from build123d import *

# Parameters (mm, degrees)
BASE_BLOCK_SKETCH_W     = 90
BASE_BLOCK_SKETCH_H     = 33
BASE_BLOCK_DEPTH        = 32
BOTTOM_SLOT_SKETCH_W    = 26
BOTTOM_SLOT_SKETCH_H    = 14
BOTTOM_SLOT_DEPTH       = 102.05938848
SUPPORT_UPRIGHTS_DEPTH  = 90
CENTRE_RECESS_DEPTH     = 128.027556066
CRADLE_ARC_CUT_DEPTH    = 128.027556066
UPRIGHT_U_SLOT_SKETCH_W = 28
UPRIGHT_U_SLOT_SKETCH_H = 16
UPRIGHT_U_SLOT_DEPTH    = 45


with BuildPart() as part:
    # Base Block Sketch → Base Block (new, symmetric)
    with BuildSketch(Plane.XY):
        with Locations((45, 16.5)):
            Rectangle(BASE_BLOCK_SKETCH_W, BASE_BLOCK_SKETCH_H)
    extrude(amount=BASE_BLOCK_DEPTH, both=True)

    # Bottom Slot Sketch → Bottom Slot (cut, through all)
    with BuildSketch(Plane(origin=(90, 0, 0), x_dir=(0, 0, -1), z_dir=(1, 0, 0))):
        with Locations((0, 7)):
            Rectangle(BOTTOM_SLOT_SKETCH_W, BOTTOM_SLOT_SKETCH_H)
    extrude(amount=-BOTTOM_SLOT_DEPTH, mode=Mode.SUBTRACT)

    # Support Uprights Sketch → Support Uprights (add)
    with BuildSketch(Plane(origin=(90, 0, 0), x_dir=(0, 0, -1), z_dir=(1, 0, 0))):
        Polygon((-24, 33), (24, 33), (24, 70), (8, 70), (8, 45), (-8, 45), (-8, 70), (-24, 70), align=None)
    extrude(amount=-SUPPORT_UPRIGHTS_DEPTH)

    # Centre Recess Sketch → Centre Recess (cut, through all)
    with BuildSketch(Plane.XY.offset(24)):
        Polygon((90, 70), (73.829610801, 70), (90, 33), align=None)
        Polygon((0, 33), (13.829610801, 70), (0, 70), align=None)
    extrude(amount=-CENTRE_RECESS_DEPTH, mode=Mode.SUBTRACT)

    # Cradle Arc Sketch → Cradle Arc Cut (cut, through all)
    with BuildSketch(Plane(origin=(0, 0, -24), x_dir=(-1, 0, 0), z_dir=(0, 0, -1))):
        with BuildLine():
            Line((-23.829610801, 70), (-63.829610801, 70))
            ThreePointArc((-63.829610801, 70), (-43.829610801, 50), (-23.829610801, 70))
        make_face()
    extrude(amount=-CRADLE_ARC_CUT_DEPTH, mode=Mode.SUBTRACT)

    # Upright U-Slot Sketch → Upright U-Slot (cut)
    with BuildSketch(Plane(origin=(0, 70, 0), x_dir=(1, 0, 0), z_dir=(0, 1, 0))):
        with Locations((45, 24)):
            Rectangle(UPRIGHT_U_SLOT_SKETCH_W, UPRIGHT_U_SLOT_SKETCH_H)
        with Locations((45, -24)):
            Rectangle(UPRIGHT_U_SLOT_SKETCH_W, UPRIGHT_U_SLOT_SKETCH_H)
    extrude(amount=-UPRIGHT_U_SLOT_DEPTH, mode=Mode.SUBTRACT)


solid = part.part
Could you check a few things on this model? Use its own coordinates, in mm. A direction names the side the tool comes from. Give positions to 0.01 mm unless a question says otherwise; leave off trailing zeros. Loops run counter-clockwise (first coordinate to the right, second up) from the corner with the lowest first, then second, coordinate; pieces in that order, holes last. Notation, with made-up numbers: (-7, -31) -> (10, -31) arc R15 cw to (10, -22) -> close; hole circle Ø11 at (15, 60.5). An arc over 180 degrees is marked (long way). Answer as CSV lines item,"result". Start each with the question number.
(1) If we section it at C-C on z = -2: Write out the boundary of the cut face in (x, y).
(2) If we section it at A-A on y = 11.5: Write out the boundary of the cut face in (x, z).
(3) If we section it at B-B on x = 18: Write out the boundary of the cut face in (y, z).
(4) I need wall thicknesses on probe 1 along Z at (x, y) = (10, 53); probe 2 along Y at (x, z) = (62.5, 6.5); probe 3 along Z at (x, y) = (66, 41). Which ranges of each line are inside material? Lowest first, please.
(5) I'm going to push flat-ended pins straight in: pin 1 Ø8 at (y, z) = (38, -26) entering from +X; pin 2 Ø4 at (x, z) = (56, 12) entering from +Y; pin 3 Ø8.5 at (x, y) = (44.5, 44) entering from +Z. Where does each tip first touch, or does it pass through?
(6) Which directions (+Z, -Z, +X, -X, +Y, -Y) give clear straight access to the entire face, cutting with the end or side of a thin tool? Please do faces 5 (the flat face through (74, 33, -28)), 6 (the flat face through (19, 48, 24)), 7 (the flat face through (59, 38, -22)), 8 (the flat face through (31, 37, 21)), 9 (the flat face through (46, 14, 0)).
(7) If we section it at D-D on y = 53: Write out the boundary of the cut face in (x, z), then the cut area to 3 significant figures.
(8) We'd pull the mould along X, two halves only. Please class faces 1 (the flat face through (85.395, 43.537, 0.336)), 2 (the flat face through (45, 25, -24)), 3 (the flat face through (3.745, 43.019, 0.336)), 4 (the flat face through (15, 33, -28)): released by +X, released by -X, zero draft, split by the parting line, or undercut.
Computed:
1,outline,"(0, 14) -> (90, 14) -> (90, 33) -> (84.76, 45) -> (4.49, 45) -> (0, 33) -> close"
2,outline,"(0, -32) -> (90, -32) -> (90, -13) -> (0, -13) -> close; (0, 13) -> (90, 13) -> (90, 32) -> (0, 32) -> close"
3,outline,"(0, -32) -> (33, -32) -> (33, -24) -> (70, -24) -> (70, -8) -> (45, -8) -> (45, 8) -> (70, 8) -> (70, 24) -> (33, 24) -> (33, 32) -> (0, 32) -> (0, 13) -> (14, 13) -> (14, -13) -> (0, -13) -> close"
4,probe 1,"z = -24 to -8, 8 to 24"
4,probe 2,"y = 14 to 45"
4,probe 3,"z = -24 to 24"
5,pin 1,"stops at x = 89.33"
5,pin 2,"stops at y = 55.89"
5,pin 3,"stops at z = 16"
6,face 5,"-Z, +X, -X, +Y"
6,face 6,"+Z, +X, -X, +Y"
6,face 7,"-Z, +Y"
6,face 8,"+Z, +Y"
6,face 9,"+X, -X, -Y"
7,outline,"(7.48, -24) -> (31, -24) -> (31, -16) -> (33.29, -16) -> (33.29, -8) -> (7.48, -8) -> close; (7.48, 8) -> (33.29, 8) -> (33.29, 16) -> (31, 16) -> (31, 24) -> (7.48, 24) -> close; (54.37, -16) -> (59, -16) -> (59, -24) -> (81.26, -24) -> (81.26, -8) -> (54.37, -8) -> close; (54.37, 8) -> (81.26, 8) -> (81.26, 24) -> (59, 24) -> (59, 16) -> (54.37, 16) -> close"
7,area,"1,580 mm2"
8,face 1,"released by +X"
8,face 2,"undercut"
8,face 3,"released by -X"
8,face 4,"zero draft"
